Read the model definition and answer for the solid it produces. Units are mm, in the model's axes. A direction names the side the tool comes from. Give positions to 0.01 mm unless a question says otherwise; leave off trailing zeros. Write each loop counter-clockwise with the first axis right and the second up, starting at its lowest first coordinate (ties: lowest second). Pieces come first, ordered by that corner, then holes.
```python
from build123d import *

# Parameters (mm, degrees)
SKETCH_1_W          = 480
SKETCH_1_H          = 400
EXTRUDE_1_DEPTH     = 2
SKETCH_2_R          = 3
CUT_EXTRUDE_1_DEPTH = 313.416388815
FILLET_1_R          = 5
SKETCH_3_W          = 430
SKETCH_3_H          = 350
CUT_EXTRUDE_2_DEPTH = 313.416388815
FILLET_2_R          = 30


with BuildPart() as part:
    # 草图1 → 凸台-拉伸1 (new body)
    with BuildSketch(Plane(origin=(0, 0, 0), x_dir=(0, 0, -1), z_dir=(1, 0, 0))):
        Rectangle(SKETCH_1_W, SKETCH_1_H)
    extrude(amount=EXTRUDE_1_DEPTH)

    # 草图2 → 切除-拉伸1 (cut, through all)
    with BuildSketch(Plane(origin=(2, 0, 0), x_dir=(0, 0, -1), z_dir=(1, 0, 0))):
        with Locations((-225, 185)):
            Circle(SKETCH_2_R)
        with Locations((225, 185)):
            Circle(SKETCH_2_R)
        with Locations((-225, -185)):
            Circle(SKETCH_2_R)
        with Locations((225, -185)):
            Circle(SKETCH_2_R)
    extrude(amount=-CUT_EXTRUDE_1_DEPTH, mode=Mode.SUBTRACT)

    # 圆角1
    fillet_1_edges = [part.edges().sort_by_distance(p)[0] for p in [
        (1, 200, 240),
        (1, 200, -240),
        (1, -200, -240),
        (1, -200, 240),
    ]]
    fillet(fillet_1_edges, radius=FILLET_1_R)

    # 草图3 → 切除-拉伸2 (cut, through all)
    with BuildSketch(Plane(origin=(2, 0, 0), x_dir=(0, 0, -1), z_dir=(1, 0, 0))):
        Rectangle(SKETCH_3_W, SKETCH_3_H)
    extrude(amount=-CUT_EXTRUDE_2_DEPTH, mode=Mode.SUBTRACT)

    # 圆角2
    fillet_2_edges = [part.edges().sort_by_distance(p)[0] for p in [
        (1, -175, 215),
        (1, 175, 215),
        (1, 175, -215),
        (1, -175, -215),
    ]]
    fillet(fillet_2_edges, radius=FILLET_2_R)


solid = part.part
```
Item 1: Which of the six approach directions +Z, -Z, +X, -X, +Y, -Y give full straight-line access (tool end or side, diameter ignored) to faces 1 (the flat face through (2, -177, 19)), 2 (the cylindrical face through (0.986, 165.979, -206.445))?
Result set:
face 1: +Z, -Z, +X, +Y, -Y
face 2: +X, -X
Item 2: Determine the mould class of faces 3 (the flat face through (0, -177, 19)), 4 (the cylindrical face through (0.986, 166.445, 205.979)) for opening direction Z: pulls with the +Z half, pulls with the -Z half, needs draft (parallel to the pull), parting line crosses it, or undercut.
Result set:
face 3: needs draft
face 4: undercut
Item 3: Section A-A (y = -114.5) is taken. Write down the section's boundary in (x, z).
Result set:
outline: (0, -240) - (2, -240) - (2, -215) - (0, -215) - close; (0, 215) - (2, 215) - (2, 240) - (0, 240) - close
Item 4: Section B-B (z = 154) is taken. Write down the section's boundary in (x, y).
Result set:
outline: (0, -200) - (2, -200) - (2, -175) - (0, -175) - close; (0, 175) - (2, 175) - (2, 200) - (0, 200) - close
Item 5: Each of these flat-tipped pins is pushed along its axis until it touches: pin 1 Ø9.5 at (y, z) = (185, 225) entering from +X; pin 2 Ø5.5 at (y, z) = (-185, -225) entering from +X. Where does it stop, or does it pass through?
Result set:
pin 1: stops at x = 2
pin 2: passes through
Item 6: Section C-C (x = 1) is taken. Write down the section's boundary in (y, z).
Result set:
outline: (-200, -235) arc R5 ccw to (-195, -240) - (195, -240) arc R5 ccw to (200, -235) - (200, 235) arc R5 ccw to (195, 240) - (-195, 240) arc R5 ccw to (-200, 235) - close; hole circle Ø6 at (-185, -225); hole circle Ø6 at (-185, 225); hole (-175, -185) arc R30 ccw to (-145, -215) - (145, -215) arc R30 ccw to (175, -185) - (175, 185) arc R30 ccw to (145, 215) - (-145, 215) arc R30 ccw to (-175, 185) - close; hole circle Ø6 at (185, -225); hole circle Ø6 at (185, 225)
Item 7: Find the intervals of material crossed by line 1 along Z through (x, y) = (0.55, 185); line 2 along Y through (x, z) = (0.65, 225); line 3 along Y through (x, z) = (0.4, -173.5), in increasing order.
Result set:
line 1: z = -240 to -228, -222 to 222, 228 to 240
line 2: y = -200 to -188, -182 to 182, 188 to 200
line 3: y = -200 to -175, 175 to 200
